```python
from build123d import *

# Parameters (mm, degrees)
FEET_AND_UPRIGHTS_CUT_DEPTH          = 99.994949528
FEET_AND_UPRIGHTS_CUT_DEPTH_BACK     = 99.994949528
FEET_AND_UPRIGHTS_PROFILE_SKETCH_W   = 29.409363616
FEET_AND_UPRIGHTS_PROFILE_SKETCH_H   = 32
FEET_AND_UPRIGHTS_PROFILE_SKETCH_W_2 = 50
FEET_AND_UPRIGHTS_PROFILE_SKETCH_H_2 = 20
BASE_ARCH_CUT_DEPTH                  = 99.994949528
BASE_ARCH_CUT_DEPTH_BACK             = 99.994949528
CRADLE_SADDLES_CUT_DEPTH             = 99.994949528
CRADLE_SADDLES_CUT_DEPTH_BACK        = 99.994949528
WEB_WINDOW_CUT_DEPTH                 = 99.994949528
WEB_WINDOW_CUT_DEPTH_BACK            = 99.994949528
WEB_WINDOW_SKETCH_W                  = 24
WEB_WINDOW_SKETCH_H                  = 20


with BuildPart() as part:
    # Base Profile Sketch → Tapered Block Loft section 0
    with BuildSketch(Plane(origin=(0, 0, 0), x_dir=(1, 0, 0), z_dir=(0, 1, 0))):
        with BuildLine():
            Line((-50, -30), (50, -30))
            Line((50, -30), (50, 30))
            Line((50, 30), (-50, 30))
            Line((-50, 30), (-50, -30))
        make_face()
    # Top Profile Sketch → Tapered Block Loft section 1
    with BuildSketch(Plane(origin=(0, 80, 0), x_dir=(1, 0, 0), z_dir=(0, 1, 0))):
        with BuildLine():
            Line((-41, -20), (41, -20))
            Line((41, -20), (41, 20))
            Line((41, 20), (-41, 20))
            Line((-41, 20), (-41, -20))
        make_face()
    loft()

    # Feet and Uprights Profile Sketch → Feet and Uprights Cut (cut, two sides: drawn at the far end of the back side and taken through both)
    with BuildSketch(Plane.XY.offset(-FEET_AND_UPRIGHTS_CUT_DEPTH_BACK)):
        with Locations((-44.704681808, 28)):
            Rectangle(FEET_AND_UPRIGHTS_PROFILE_SKETCH_W, FEET_AND_UPRIGHTS_PROFILE_SKETCH_H)
        with Locations((0, 70)):
            Rectangle(FEET_AND_UPRIGHTS_PROFILE_SKETCH_W_2, FEET_AND_UPRIGHTS_PROFILE_SKETCH_H_2)
        with Locations((44.704681808, 28)):
            Rectangle(FEET_AND_UPRIGHTS_PROFILE_SKETCH_W, FEET_AND_UPRIGHTS_PROFILE_SKETCH_H)
    extrude(amount=FEET_AND_UPRIGHTS_CUT_DEPTH + FEET_AND_UPRIGHTS_CUT_DEPTH_BACK, mode=Mode.SUBTRACT)

    # Base Arch Sketch → Base Arch Cut (cut, two sides: drawn at the far end of the back side and taken through both)
    with BuildSketch(Plane(origin=(0, 0, 0), x_dir=(0, 0, -1), z_dir=(1, 0, 0)).offset(-BASE_ARCH_CUT_DEPTH_BACK)):
        with BuildLine():
            Line((-10, 80), (10, 80))
            ThreePointArc((10, 80), (0, 70), (-10, 80))
        make_face()
    extrude(amount=BASE_ARCH_CUT_DEPTH + BASE_ARCH_CUT_DEPTH_BACK, mode=Mode.SUBTRACT)

    # Cradle Saddles Sketch → Cradle Saddles Cut (cut, two sides: drawn at the far end of the back side and taken through both)
    with BuildSketch(Plane(origin=(0, 0, 0), x_dir=(0, 0, -1), z_dir=(1, 0, 0)).offset(-CRADLE_SADDLES_CUT_DEPTH_BACK)):
        with BuildLine():
            Line((-15, 12), (-15, 0))
            Line((-15, 0), (15, 0))
            Line((15, 0), (15, 12))
            ThreePointArc((15, 12), (0, 27), (-15, 12))
        make_face()
    extrude(amount=CRADLE_SADDLES_CUT_DEPTH + CRADLE_SADDLES_CUT_DEPTH_BACK, mode=Mode.SUBTRACT)

    # Web Window Sketch → Web Window Cut (cut, two sides: drawn at the far end of the back side and taken through both)
    with BuildSketch(Plane.XY.offset(-WEB_WINDOW_CUT_DEPTH_BACK)):
        with Locations((0, 40)):
            Rectangle(WEB_WINDOW_SKETCH_W, WEB_WINDOW_SKETCH_H)
    extrude(amount=WEB_WINDOW_CUT_DEPTH + WEB_WINDOW_CUT_DEPTH_BACK, mode=Mode.SUBTRACT)


solid = part.part
```
Geometry check sheet. Reference: the model listing, model coordinates, mm. A direction names the side the tool comes from. Coordinates: 2 decimals unless noted, no trailing zeros.
Item 1: Scan lines: line 1 along Y through (x, z) = (5.5, 18); line 2 along X through (y, z) = (33.5, 5); line 3 along X through (y, z) = (28, 22). Record each from-to range of solid material in increasing order.
Item 2: Depth check by flat-ended pin: pin 1 (3 mm diameter, centred on x = 18, z = 10.5, fed in from -Y); pin 2 (13.5 mm diameter, centred on x = -2, z = 5, fed in from +Y); pin 3 (15 mm diameter, centred on x = -42, z = 19, fed in from +Y); pin 4 (10 mm diameter, centred on y = 30, z = -18.5, fed in from +X). Enter the tip coordinate at first touch or a pass-through.
Item 3: Section check A-A (x = -37.5). Count the separate pieces of the cut face and the enclosed holes in it, plus the area to 3 significant figures.
Item 4: Tool access check on faces 1 (the flat face through (0, 50, 0)), 2 (the flat face through (-25, 68, 0)), 3 (the flat face through (39, 12, -22)), 4 (the flat face through (-39, 12, -22)). Record the directions out of +Z, -Z, +X, -X, +Y, -Y that give a thin tool (end or side, any length) a straight path to the whole face; none if there is none.
Item 5: Mould release check, pull along Y, two halves, no side actions. Record for faces 5 (the flat face through (-1, 0, -24)), 6 (the flat face through (-1, 6, 15)), 7 (the flat face through (39, 12, 22)): released by +Y, released by -Y, zero draft, split by the parting line, or undercut.
Check sheet entries:
1. line 1: y = 0 to 30, 50 to 60
1. line 2: x = -30 to -12, 12 to 30
1. line 3: x = -30 to 30
2. pin 1: stops at y = 21
2. pin 2: stops at y = 60
2. pin 3: stops at y = 80
2. pin 4: stops at x = 30
3. separate pieces: 3
3. enclosed holes: 0
3. area: 1,790 mm2
4. face 1: +Z, -Z
4. face 2: +Z, -Z, +Y
4. face 3: +Z, -Z, +X
4. face 4: +Z, -Z, -X
5. face 5: released by -Y
5. face 6: zero draft
5. face 7: undercut
